```python
from build123d import *

# Parameters (mm, degrees)
SKETCH_1_W          = 60
SKETCH_1_H          = 60
EXTRUDE_1_DEPTH     = 30
SHELL_1_T           = -1.5
SKETCH_5_W          = 1.5
SKETCH_5_H          = 60
EXTRUDE_3_DEPTH     = 10
SKETCH_6_W          = 1.5
SKETCH_6_H          = 60
EXTRUDE_4_DEPTH     = 10
CUT_EXTRUDE_3_REACH = 80.102
SKETCH_7_W          = 20
SKETCH_7_H          = 15
FILLET_1_R          = 5
FILLET_2_R          = 5
CUT_EXTRUDE_4_REACH = 80.102
SKETCH_8_R          = 11.5
FILLET_3_R          = 1
SKETCH_9_R          = 3
CUT_EXTRUDE_5_DEPTH = 77.956156349


with BuildPart() as part:
    # 草图1 → 凸台-拉伸1 (new, symmetric)
    with BuildSketch(Plane.XY):
        Rectangle(SKETCH_1_W, SKETCH_1_H)
    extrude(amount=EXTRUDE_1_DEPTH, both=True)

    # 抽壳1
    shell_1_openings = [part.faces().sort_by_distance(p)[0] for p in [
        (0, 0, -30),
    ]]
    offset(amount=SHELL_1_T, openings=shell_1_openings, kind=Kind.INTERSECTION)

    # 草图5 → 凸台-拉伸3 (add)
    with BuildSketch(Plane(origin=(30, 0, 0), x_dir=(0, 0, -1), z_dir=(1, 0, 0))):
        with Locations((29.25, 0)):
            Rectangle(SKETCH_5_W, SKETCH_5_H)
    extrude(amount=EXTRUDE_3_DEPTH)

    # 草图6 → 凸台-拉伸4 (add)
    with BuildSketch(Plane.ZY.offset(30)):
        with Locations((-29.25, 0)):
            Rectangle(SKETCH_6_W, SKETCH_6_H)
    extrude(amount=EXTRUDE_4_DEPTH)

    # 草图7 → 切除-拉伸3 (cut, up to next)
    with BuildSketch(Plane.XZ.offset(30), mode=Mode.PRIVATE) as cut_extrude_3_sk1:
        with Locations((0, -22.5)):
            Rectangle(SKETCH_7_W, SKETCH_7_H)
    cut_extrude_3_tool1 = extrude(cut_extrude_3_sk1.sketch, amount=-CUT_EXTRUDE_3_REACH, mode=Mode.PRIVATE) & part.part
    add(cut_extrude_3_tool1.solids().sort_by_distance((0, -30, -22.5))[0], mode=Mode.SUBTRACT)

    # 圆角1
    fillet_1_edges = [part.edges().sort_by_distance(p)[0] for p in [
        (10, -29.25, -15),
        (-10, -29.25, -15),
    ]]
    fillet(fillet_1_edges, radius=FILLET_1_R)

    # 圆角2
    fillet_2_edges = [part.edges().sort_by_distance(p)[0] for p in [
        (40, 30, -29.25),
        (40, -30, -29.25),
        (-40, -30, -29.25),
        (-40, 30, -29.25),
    ]]
    fillet(fillet_2_edges, radius=FILLET_2_R)

    # 草图8 → 切除-拉伸4 (cut, up to next)
    with BuildSketch(Plane(origin=(0, 30, 0), x_dir=(1, 0, 0), z_dir=(0, 1, 0)), mode=Mode.PRIVATE) as cut_extrude_4_sk1:
        with Locations(Location((0, 0, 0), (0, 0, 270))):
            Circle(SKETCH_8_R)
    cut_extrude_4_tool1 = extrude(cut_extrude_4_sk1.sketch, amount=-CUT_EXTRUDE_4_REACH, mode=Mode.PRIVATE) & part.part
    add(cut_extrude_4_tool1.solids().sort_by_distance((0, 30, 0))[0], mode=Mode.SUBTRACT)

    # 圆角3
    fillet_3_edges = [part.edges().sort_by_distance(p)[0] for p in [
        (-30, 0, 30),
        (0, -30, 30),
        (30, 0, 30),
        (0, 30, 30),
        (30, -30, 0.75),
        (-30, -30, 0.75),
        (-30, 30, 0.75),
        (30, 30, 0.75),
    ]]
    fillet(fillet_3_edges, radius=FILLET_3_R)

    # 草图9 → 切除-拉伸5 (cut, through all)
    with BuildSketch(Plane.XY.offset(-28.5)):
        with Locations((35, -15)):
            Circle(SKETCH_9_R)
        with Locations((35, 15)):
            Circle(SKETCH_9_R)
    cut_extrude_5 = extrude(amount=-CUT_EXTRUDE_5_DEPTH, mode=Mode.SUBTRACT)

    # 镜向1: 切除-拉伸5 across plane
    add(cut_extrude_5.mirror(Plane(origin=(0, 0, 0), x_dir=(0, 0, 1), z_dir=(1, 0, 0))), mode=Mode.SUBTRACT)


solid = part.part
```
Check sheet for the modelled part. Datum: model origin and axes. Units: mm. A direction names the side the tool comes from. Round coordinates to 2 decimals unless told otherwise and drop trailing zeros. Write each loop counter-clockwise with the first axis right and the second up, starting at its lowest first coordinate (ties: lowest second). Pieces come first, ordered by that corner, then holes. Notation, with made-up numbers: (50, 50.25) -> (59, 50.25) arc R30 cw to (59, 85.25) -> close; hole circle Ø7 at (-26.75, 42.25). An arc over 180 degrees is marked (long way). One line per question, with ' | ' between items. Start each with the question number.
1. Set-up check for faces 1 (the face through (-9, -29, -17)), 2 (the face through (-30, 0, 1)), 3 (the face through (28.5, 0, 0)): record each of +Z, -Z, +X, -X, +Y, -Y from which the full face is reachable in a straight line by a thin tool's end or side.
2. Depth check by flat-ended pin: pin 1 (6 mm diameter, centred on x = -5.5, y = 13, fed in from -Z); pin 2 (8 mm diameter, centred on y = -15.5, z = 21, fed in from -X); pin 3 (1.6 mm diameter, centred on x = 1, y = -29.5, fed in from -Z). Enter the tip coordinate at first touch or a pass-through.
3. Release check for a two-part mould opening along Z. For faces 4 (the face through (9, -29, -17)), 5 (the face through (0, 0, 30)), 6 (the face through (9.7, 29.26, 6.18)) record: +Z half, -Z half, draft (parallel to the pull), parting line (faces both ways), or undercut.
4. Sectioned sample at B-B, the plane y = 15. Record the cut outline in (x, z), then the cut area to 3 significant figures.
5. Sectioned sample at A-A, the plane x = 0. Record the cut outline in (y, z).
6. Scan lines: line 1 along Y through (x, z) = (-35, -28.75); line 2 along Y through (x, z) = (-16, 17.5). Record each from-to range of solid material in increasing order. Write a range as from..to.
7. Sectioned sample at C-C, the plane z = 22. Record the cut outline in (x, y), then the cut area to 3 significant figures.
8. Sectioned sample at D-D, the plane y = 21. Record the cut outline in (x, z), then the cut area to 3 significant figures.
Taken from the geometry:
1) face 1: -Z, -Y | face 2: +Z, -X, +Y, -Y | face 3: -Z
2) pin 1: stops at z = 28.5 | pin 2: stops at x = -30 | pin 3: stops at z = -15
3) face 4: -Z half | face 5: +Z half | face 6: undercut
4) outline: (-40, -30) -> (-38, -30) -> (-38, -28.5) -> (-40, -28.5) -> close; (-32, -30) -> (-28.5, -30) -> (-28.5, 28.5) -> (28.5, 28.5) -> (28.5, -30) -> (32, -30) -> (32, -28.5) -> (30, -28.5) -> (30, 29) arc R1 ccw to (29, 30) -> (-29, 30) arc R1 ccw to (-30, 29) -> (-30, -28.5) -> (-32, -28.5) -> close; (38, -30) -> (40, -30) -> (40, -28.5) -> (38, -28.5) -> close | area: 277 mm^2
5) outline: (-30, -15) -> (-28.5, -15) -> (-28.5, 28.5) -> (28.5, 28.5) -> (28.5, 11.5) -> (30, 11.5) -> (30, 29) arc R1 ccw to (29, 30) -> (-29, 30) arc R1 ccw to (-30, 29) -> close; (28.5, -30) -> (30, -30) -> (30, -11.5) -> (28.5, -11.5) -> close
6) line 1: y = -30..-18, -12..12, 18..30 | line 2: y = -30..-28.5, 28.5..30
7) outline: (-30, -29) arc R1 ccw to (-29, -30) -> (29, -30) arc R1 ccw to (30, -29) -> (30, 29) arc R1 ccw to (29, 30) -> (-29, 30) arc R1 ccw to (-30, 29) -> close; hole (-28.5, -28.5) -> (28.5, -28.5) -> (28.5, 28.5) -> (-28.5, 28.5) -> close | area: 350 mm^2
8) outline: (-40, -30) -> (-28.5, -30) -> (-28.5, 28.5) -> (28.5, 28.5) -> (28.5, -30) -> (40, -30) -> (40, -28.5) -> (30, -28.5) -> (30, 29) arc R1 ccw to (29, 30) -> (-29, 30) arc R1 ccw to (-30, 29) -> (-30, -28.5) -> (-40, -28.5) -> close | area: 295 mm^2
